```python
from build123d import *


with BuildPart() as part:
    # 草图1 → 旋转1 (revolve)
    with BuildSketch(Plane.XY, mode=Mode.PRIVATE) as revolve_1_sk:
        with BuildLine():
            Line((0, -19.516129032), (24, -19.516129032))
            Line((24, -19.516129032), (24, -16.516129032))
            Line((24, -16.516129032), (30, -16.516129032))
            Line((30, -16.516129032), (30, -11.516129032))
            ThreePointArc((30, -11.516129032), (26.485281374, -3.030847658), (18, 0.483870968))
            Line((18, 0.483870968), (9.2, 0.483870968))
            Line((9.2, 0.483870968), (8.089553055, 2.611524037))
            Line((8.089553055, 2.611524037), (8.089553055, 4.611524037))
            Line((8.089553055, 4.611524037), (11.089553055, 4.611524037))
            Line((11.089553055, 4.611524037), (11.089553055, 12.611524037))
            Line((11.089553055, 12.611524037), (6.089553055, 12.611524037))
            Line((6.089553055, 12.611524037), (6.089553055, 25.611524037))
            Line((6.089553055, 25.611524037), (11.089553055, 25.611524037))
            Line((11.089553055, 25.611524037), (11.089553055, 33.611524037))
            ThreePointArc((11.089553055, 33.611524037), (12.752211126, 34.669644876), (13.399553055, 36.531095923))
            Line((13.399553055, 36.531095923), (18.3, 64.483870968))
            Line((18.3, 64.483870968), (0, 64.483870968))
            Line((0, 64.483870968), (0, -19.516129032))
        make_face()
    revolve(revolve_1_sk.sketch.rotate(Axis((0, 0, 0), (0, 1, 0)), 90), axis=Axis((0, 0, 0), (0, 1, 0)))


solid = part.part
```
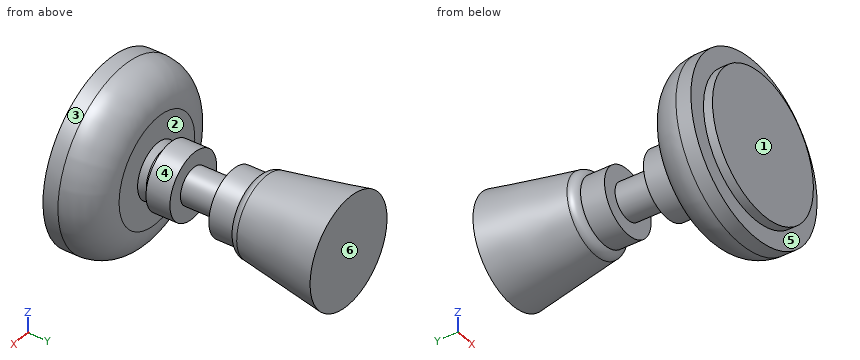
Input: part model. Units: mm. Frame: model coordinates. Face numbers are marked on the shaded views. A direction names the side the tool comes from. Coordinates: 2 decimals unless noted, no trailing zeros. Write each loop counter-clockwise with the first axis right and the second up, starting at its lowest first coordinate (ties: lowest second). Pieces come first, ordered by that corner, then holes. Notation, with made-up numbers: (-26, -24.5) - (14, -24.5) arc R28 cw to (14, 9.5) - close; hole circle Ø8 at (-23.5, -30.5). An arc over 180 degrees is marked (long way). Put each result on its own line as item: value. Start each with the question number.
1) Reachability of the marked faces 4, 5 and 6 from +Z, -Z, +X, -X, +Y, -Y: full face, straight path, thin tool, end or side. Return the list, or none.
2) Cut plane C-C (y = 27). Return the cut outline in (x, z), plus the area to 3 significant figures.
3) Cut plane D-D (y = 53). Return the cut outline in (x, z).
4) Mould query, pull axis Y, two halves, no side actions, for the marked faces 1, 2 and 3. Classes: pulls with the +Y half, pulls with the -Y half, needs draft (parallel to the pull), parting line crosses it, or undercut.
5) Ray query, L1, parallel to X at y = -4, z = -7; L2, parallel to Y at x = -14.5, z = -18.5; L3, parallel to X at y = -12.5, z = -9. Return the intervals inside material, ascending.
6) Contact query for flat-ended pins moving along their axis: pin 1 (8 mm diameter, centred on y = 55.5, z = 13.5, fed in from +X); pin 2 (4 mm diameter, centred on x = 7.5, y = 13, fed in from -Z); pin 3 (1 mm diameter, centred on x = 15, y = 36.5, fed in from -Z); pin 4 (12 mm diameter, centred on y = 37.5, z = 9, fed in from +X). Output: stop coordinate, or through.
Resolved:
1. face 4: none
1. face 5: -Y
1. face 6: +Z, -Z, +X, -X, +Y
2. outline: circle Ø22.18 at (0, 0)
2. area: 386 mm2
3. outline: circle Ø32.57 at (0, 0)
4. face 1: pulls with the -Y half
4. face 2: undercut
4. face 3: needs draft
5. L1: x = -26.44 to 26.44
5. L2: y = -19.52 to -0.85
5. L3: x = -28.62 to 28.62
6. pin 1: stops at x = 13.89
6. pin 2: stops at z = -9.61
6. pin 3: passes through
6. pin 4: stops at x = 13.57
